Geometry: final body of the model. Coordinates: model frame, mm. A direction names the side the tool comes from. Coordinates: 2 decimals unless noted, no trailing zeros. Loops run counter-clockwise (first coordinate to the right, second up) from the corner with the lowest first, then second, coordinate; pieces in that order, holes last. Notation, with made-up numbers: (24, -28) - (33, -28) arc R9 cw to (33, -20) - close; hole circle Ø5 at (80, 72.25). An arc over 180 degrees is marked (long way). Answer in a Markdown table with one row per item.
from build123d import *

# Parameters (mm, degrees)
SKETCH_1_W                = 20
SKETCH_1_H                = 30
EXTRUDE_1_DEPTH           = 20
HOLE_WIZARD_1_D           = 6.6
HOLE_WIZARD_1_CBORE_D     = 11
HOLE_WIZARD_1_CBORE_DEPTH = 6.8
HOLE_WIZARD_M4_1_D        = 3.3
CHAMFER_1_SIZE            = 2


with BuildPart() as part:
    # 草图1 → 凸台-拉伸1 (new body)
    with BuildSketch(Plane.XY):
        Rectangle(SKETCH_1_W, SKETCH_1_H)
    extrude(amount=EXTRUDE_1_DEPTH)

    # 打孔尺寸根据内六角圆柱头螺钉的类型1 (through all)
    with Locations(Plane(origin=(3.133596483, 10.907898158, 0), x_dir=(1, 0, 0), z_dir=(0, 0, -1))):
        with Locations((-3.133596483, 17.907898158)):
            CounterBoreHole(HOLE_WIZARD_1_D / 2, HOLE_WIZARD_1_CBORE_D / 2, HOLE_WIZARD_1_CBORE_DEPTH)

    # M4 螺纹孔1 (through all)
    with Locations(Plane.ZY.offset(10)):
        with Locations((5, 7)):
            Hole(HOLE_WIZARD_M4_1_D / 2)

    # 倒角1
    chamfer_1_edges = [part.edges().sort_by_distance(p)[0] for p in [
        (10, -15, 10),
        (-10, -15, 10),
        (-10, 15, 10),
        (10, 15, 10),
    ]]
    chamfer(chamfer_1_edges, length=CHAMFER_1_SIZE)


solid = part.part
(1) First-contact query: pin 1 Ø9 at (x, y) = (0.5, -6) entering from -Z; pin 2 Ø2 at (x, y) = (1.5, -6) entering from -Z (3 decimals); pin 3 Ø7.5 at (x, y) = (0, -7) entering from -Z. Flat tips, straight axial feed; report the tip coordinate or a pass-through.
Verdict:
| item | result |
|---|---|
| pin 1 | stops at z = 0 |
| pin 2 | passes through |
| pin 3 | stops at z = 6.8 |
(2) Pull-direction query (Y, two-part tool) for faces 3 (the face through (-9, -14, 10)), 4 (the face through (4, -7, 6.8)), 5 (the face through (10, 0, 10)); classes: pulls with the +Y half, pulls with the -Y half, needs draft (parallel to the pull), parting line crosses it, or undercut.
Verdict:
| item | result |
|---|---|
| face 3 | pulls with the -Y half |
| face 4 | undercut |
| face 5 | needs draft |
(3) Cut plane C-C on z = 5. Output: boundary loops of the cut face in (x, y), then the cut area to 3 significant figures.
Verdict:
| item | result |
|---|---|
| outline | (-10, -13) - (-8, -15) - (8, -15) - (10, -13) - (10, 5.35) - (-10, 5.35) - close; (-10, 8.65) - (10, 8.65) - (10, 13) - (8, 15) - (-8, 15) - (-10, 13) - close; hole circle Ø11 at (0, -7) |
| area | 431 mm² |
(4) Cut plane D-D on z = 1.75. Output: boundary loops of the cut face in (x, y).
Verdict:
| item | result |
|---|---|
| outline | (-10, -13) - (-8, -15) - (8, -15) - (10, -13) - (10, 13) - (8, 15) - (-8, 15) - (-10, 13) - close; hole circle Ø11 at (0, -7) |
(5) Cut plane B-B on x = 0. Output: boundary loops of the cut face in (y, z).
Verdict:
| item | result |
|---|---|
| outline | (-15, 0) - (-12.5, 0) - (-12.5, 6.8) - (-10.3, 6.8) - (-10.3, 20) - (-15, 20) - close; (-3.7, 6.8) - (-1.5, 6.8) - (-1.5, 0) - (15, 0) - (15, 20) - (-3.7, 20) - close; hole circle Ø3.3 at (7, 5) |
(6) Access query for faces 1 (the face through (0, 0, 20)), 2 (the face through (-1.19, -1.63, 3.35)). Directions: +Z, -Z, +X, -X, +Y, -Y. A direction counts if a zero-diameter tool reaches every point of the face in a straight line with its end or side. Return the directions, or none.
Verdict:
| item | result |
|---|---|
| face 1 | +Z, +X, -X, +Y, -Y |
| face 2 | -Z |
(7) Ray query, probe 1 along Y at (x, z) = (0, 11.25); probe 2 along Y at (x, z) = (0, 5.25); probe 3 along Z at (x, y) = (1.5, -10). Return the intervals inside material, ascending.
Verdict:
| item | result |
|---|---|
| probe 1 | y = -15 to -10.3, -3.7 to 15 |
| probe 2 | y = -15 to -12.5, -1.5 to 5.37, 8.63 to 15 |
| probe 3 | z = 6.8 to 20 |
(8) Cut plane A-A on y = -7. Output: boundary loops of the cut face in (x, z), then the cut area to 3 significant figures.
Verdict:
| item | result |
|---|---|
| outline | (-10, 0) - (-5.5, 0) - (-5.5, 6.8) - (-3.3, 6.8) - (-3.3, 20) - (-10, 20) - close; (3.3, 6.8) - (5.5, 6.8) - (5.5, 0) - (10, 0) - (10, 20) - (3.3, 20) - close |
| area | 238 mm² |
